For this review, use the dimensioned drawing (mm, ordinates from the lowest corner) and the shaded views. Give positions to 0.01 mm unless a question says otherwise; leave off trailing zeros. Write each loop counter-clockwise with the first axis right and the second up, starting at its lowest first coordinate (ties: lowest second). Pieces come first, ordered by that corner, then holes. Notation, with made-up numbers: M 72,64.25 L 100,64.25 A26 ccw 100,87.25 Z; hole C 36.5,57 d1. An arc over 180 degrees is marked long. Answer in a Markdown table with one row per item.
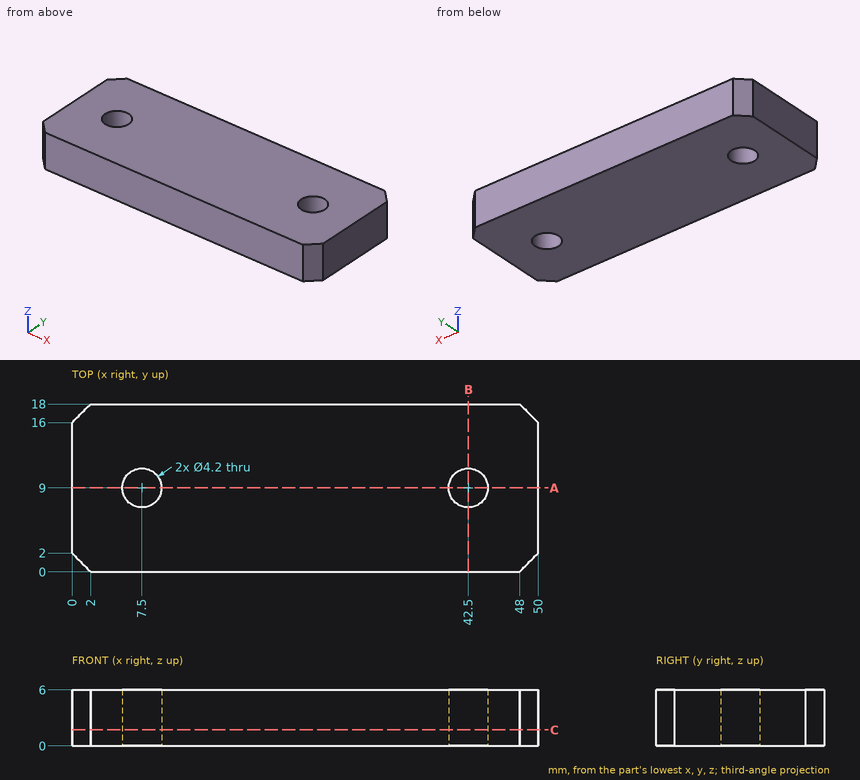
1) Add section B-B (x = 42.5). Write out the cut boundary in (y, z), and give its area (3 significant figures).
Geometry says:
| item | result |
|---|---|
| outline | M 0,0 L 6.9,0 L 6.9,6 L 0,6 Z; M 11.1,0 L 18,0 L 18,6 L 11.1,6 Z |
| area | 82.8 mm^2 |
2) Insertion check: P1, Ø5, axis at x = 37.5, y = 10, coming from the -Z side. The pin has a flat end and moves straight along its axis. Give the tip position at first contact, or say it passes through.
Geometry says:
| item | result |
|---|---|
| P1 | z = 0 |
3) Add section A-A (y = 9). Write out the cut boundary in (x, z).
Geometry says:
| item | result |
|---|---|
| outline | M 0,0 L 5.4,0 L 5.4,6 L 0,6 Z; M 9.6,0 L 40.4,0 L 40.4,6 L 9.6,6 Z; M 44.6,0 L 50,0 L 50,6 L 44.6,6 Z |
4) To check wall thickness, follow probe 1 along Y at (x, z) = (7.5, 4.6); probe 2 along X at (y, z) = (10.5, 1.95); probe 3 along Y at (x, z) = (43, 5.7). State the ranges of each line that lie inside material, in increasing order. Write a range as [from, to].
Geometry says:
| item | result |
|---|---|
| probe 1 | [0, 6.9], [11.1, 18] |
| probe 2 | [0, 6.03], [8.97, 41.03], [43.97, 50] |
| probe 3 | [0, 6.96], [11.04, 18] |
5) Add section C-C (z = 1.7). Write out the cut boundary in (x, y), and give its area (3 significant figures).
Geometry says:
| item | result |
|---|---|
| outline | M 0,2 L 2,0 L 48,0 L 50,2 L 50,16 L 48,18 L 2,18 L 0,16 Z; hole C 7.5,9 d4.2; hole C 42.5,9 d4.2 |
| area | 864 mm^2 |
